Read the model definition and answer for the solid it produces. Units are mm, in the model's axes. A direction names the side the tool comes from. Coordinates: 2 decimals unless noted, no trailing zeros. Loops run counter-clockwise (first coordinate to the right, second up) from the corner with the lowest first, then second, coordinate; pieces in that order, holes last. Notation, with made-up numbers: (52, 83.5) - (56, 83.5) arc R7 ccw to (56, 89.5) - close; hole circle Ø2 at (83, 45). An arc over 180 degrees is marked (long way). Use one line per item in the form item = value. Start each with the question number.
1) A cutting plane is placed at A-A (z = 45). Give the vertices of the cut face in (x, y).
2) This flat-tipped pin is pushed along its axis until it touches: P1, Ø2.5, axis at x = -25, z = -35, coming from the -Y side. Where does it stop, or does it pass through?
3) The mould has two halves that part along Z. Classify faces 3 (the face through (-23.21, 2.96, -21.96)), 4 (the face through (0, 3, 55)), 5 (the face through (20, 0, -1)): released by +Z, released by -Z, zero draft, split by the parting line, or undercut.
4) A cutting plane is placed at D-D (z = 5.5). Give the vertices of the cut face in (x, y), and give its area (3 significant figures).
5) Which of the six approach directions +Z, -Z, +X, -X, +Y, -Y give full straight-line access (tool end or side, diameter ignored) to faces 1 (the face through (15, 3, -47.7)), 2 (the face through (29, 3, -1))?
6) A cutting plane is placed at B-B (x = 0). Give the vertices of the cut face in (y, z), and give its area (3 significant figures).
7) Consider line 1 (X direction, y = 4.5, z = 35); line 2 (X direction, y = 2.5, z = -45); line 3 (Z direction, x = 25, y = 3.5). Determine where each line is inside the solid, lowest interval first.
8) A cutting plane is placed at C-C (y = 4.5). State how many separate pieces and enclosed holes the cut face has, and give its area (3 significant figures).
from build123d import *

# Parameters (mm, degrees)
SKETCH1_R             = 19.1
BOSS_EXTRUDE1_DEPTH   = 6
M4_TAPPED_HOLE1_D     = 3.3
M4_TAPPED_HOLE1_DEPTH = 10.1
M4_TAPPED_HOLE1_TIP   = 0.991420021
CUT_EXTRUDE1_DEPTH    = 63.465990747
M4_TAPPED_HOLE2_D     = 3.3
M4_TAPPED_HOLE2_DEPTH = 10.1
M4_TAPPED_HOLE2_TIP   = 0.991420021


with BuildPart() as part:
    # Sketch1 → Boss-Extrude1 (new body)
    with BuildSketch(Plane(origin=(0, 0, 0), x_dir=(1, 0, 0), z_dir=(0, 1, 0))):
        with BuildLine():
            Line((-23, 55), (23, 55))
            ThreePointArc((23, 55), (27.242640687, 53.242640687), (29, 49))
            Line((29, 49), (29, -49))
            ThreePointArc((29, -49), (27.242640687, -53.242640687), (23, -55))
            Line((23, -55), (-23, -55))
            ThreePointArc((-23, -55), (-27.242640687, -53.242640687), (-29, -49))
            Line((-29, -49), (-29, 49))
            ThreePointArc((-29, 49), (-27.242640687, 53.242640687), (-23, 55))
        make_face()
        with Locations(Location((0, 0, 0), (0, 0, 270))):
            Circle(SKETCH1_R, mode=Mode.SUBTRACT)
    extrude(amount=BOSS_EXTRUDE1_DEPTH)

    # M4 Tapped Hole1
    with Locations(Plane(origin=(0, 6, 0), x_dir=(1, 0, 0), z_dir=(0, 1, 0))):
        with Locations((-23.57, 23.57), (23.57, 23.57), (23.57, -23.57), (-23.57, -23.57)):
            Hole(M4_TAPPED_HOLE1_D / 2, depth=M4_TAPPED_HOLE1_DEPTH)
            with Locations((0, 0, -(M4_TAPPED_HOLE1_DEPTH + M4_TAPPED_HOLE1_TIP / 2))):  # 118° drill point
                Cone(0, M4_TAPPED_HOLE1_D / 2, M4_TAPPED_HOLE1_TIP, mode=Mode.SUBTRACT)

    # Sketch4 → Cut-Extrude1 (cut, through all)
    with BuildSketch(Plane.XZ):
        with BuildLine():
            Line((-20, 47.7), (-10, 47.7))
            ThreePointArc((-10, 47.7), (-7.3, 45), (-10, 42.3))
            Line((-10, 42.3), (-20, 42.3))
            ThreePointArc((-20, 42.3), (-22.7, 45), (-20, 47.7))
        make_face()
        with BuildLine():
            Line((20, 47.7), (10, 47.7))
            ThreePointArc((10, 47.7), (7.3, 45), (10, 42.3))
            Line((10, 42.3), (20, 42.3))
            ThreePointArc((20, 42.3), (22.7, 45), (20, 47.7))
        make_face()
        with BuildLine():
            Line((-20, -47.7), (-10, -47.7))
            ThreePointArc((-10, -47.7), (-7.3, -45), (-10, -42.3))
            Line((-10, -42.3), (-20, -42.3))
            ThreePointArc((-20, -42.3), (-22.7, -45), (-20, -47.7))
        make_face()
        with BuildLine():
            Line((20, -47.7), (10, -47.7))
            ThreePointArc((10, -47.7), (7.3, -45), (10, -42.3))
            Line((10, -42.3), (20, -42.3))
            ThreePointArc((20, -42.3), (22.7, -45), (20, -47.7))
        make_face()
    extrude(amount=-CUT_EXTRUDE1_DEPTH, mode=Mode.SUBTRACT)

    # M4 Tapped Hole2
    with Locations(Plane(origin=(0, 0, 0), x_dir=(-1, 0, 0), z_dir=(0, -1, 0))):
        with Locations((25, -35), (25, 35), (-25, 35), (-25, -35)):
            Hole(M4_TAPPED_HOLE2_D / 2, depth=M4_TAPPED_HOLE2_DEPTH)
            with Locations((0, 0, -(M4_TAPPED_HOLE2_DEPTH + M4_TAPPED_HOLE2_TIP / 2))):  # 118° drill point
                Cone(0, M4_TAPPED_HOLE2_D / 2, M4_TAPPED_HOLE2_TIP, mode=Mode.SUBTRACT)


solid = part.part
Found:
q1.outline = (-29, 0) - (-22.7, 0) - (-22.7, 6) - (-29, 6) - close; (-7.3, 0) - (7.3, 0) - (7.3, 6) - (-7.3, 6) - close; (22.7, 0) - (29, 0) - (29, 6) - (22.7, 6) - close
q2.P1 = through
q3.face_3 = undercut
q3.face_4 = released by +Z
q3.face_5 = zero draft
q4.outline = (-29, 0) - (-18.29, 0) - (-18.29, 6) - (-29, 6) - close; (18.29, 0) - (29, 0) - (29, 6) - (18.29, 6) - close
q4.area = 129 mm^2
q5.face_1 = +Y, -Y
q5.face_2 = +Z, -Z, +X, +Y, -Y
q6.outline = (0, -55) - (6, -55) - (6, -19.1) - (0, -19.1) - close; (0, 19.1) - (6, 19.1) - (6, 55) - (0, 55) - close
q6.area = 431 mm^2
q7.line_1 = -29 to -26.65, -23.35 to 23.35, 26.65 to 29
q7.line_2 = -29 to -22.7, -7.3 to 7.3, 22.7 to 29
q7.line_3 = -54.66 to -36.65, -33.35 to -24.39, -22.75 to 22.75, 24.39 to 33.35, 36.65 to 54.66
q8.separate_pieces = 1
q8.enclosed_holes = 13
q8.area = 4,830 mm^2
